from build123d import *

# Parameters (mm, degrees)
SKETCH_1_W          = 295
SKETCH_1_H          = 2005
EXTRUDE_1_DEPTH     = 30
SHELL_1_T           = -2
SKETCH_2_W          = 2
SKETCH_2_H          = 1467
EXTRUDE_2_DEPTH     = 220
SKETCH_3_R          = 4.5
CUT_EXTRUDE_1_DEPTH = 10
SKETCH_4_R          = 4.5
CUT_EXTRUDE_2_DEPTH = 116
SKETCH_5_R          = 4.5
CUT_EXTRUDE_3_DEPTH = 72
SKETCH_6_R          = 4.5
CUT_EXTRUDE_4_DEPTH = 10
CUT_EXTRUDE_START   = -10
SKETCH_7_R          = 4.5
CUT_EXTRUDE_5_DEPTH = 10
SKETCH_8_R          = 4.5
CUT_EXTRUDE_6_DEPTH = 16


with BuildPart() as part:
    # 草图1 → 凸台-拉伸1 (new body)
    with BuildSketch(Plane.XY):
        with Locations((147.5, 1002.5)):
            Rectangle(SKETCH_1_W, SKETCH_1_H)
    extrude(amount=EXTRUDE_1_DEPTH)

    # 抽壳1
    shell_1_openings = [part.faces().sort_by_distance(p)[0] for p in [
        (147.5, 1002.5, 30),
    ]]
    offset(amount=SHELL_1_T, openings=shell_1_openings, kind=Kind.INTERSECTION)

    # 草图2 → 凸台-拉伸2 (add)
    with BuildSketch(Plane.XY.offset(30)):
        with Locations((1, 773.5)):
            Rectangle(SKETCH_2_W, SKETCH_2_H)
    extrude(amount=EXTRUDE_2_DEPTH)

    # 草图3 → 切除-拉伸1 (cut)
    with BuildSketch(Plane(origin=(0, 2, 0), x_dir=(1, 0, 0), z_dir=(0, 1, 0))):
        with Locations(Location((30, -16, 0), (0, 0, 270))):
            Circle(SKETCH_3_R)
        with Locations(Location((200, -16, 0), (0, 0, 270))):
            Circle(SKETCH_3_R)
    extrude(amount=-CUT_EXTRUDE_1_DEPTH, mode=Mode.SUBTRACT)

    # 草图4 → 切除-拉伸2 (cut)
    with BuildSketch(Plane(origin=(2, 0, 0), x_dir=(0, 0, -1), z_dir=(1, 0, 0))):
        with Locations((-16, 30)):
            Circle(SKETCH_4_R)
        with Locations((-16, 180)):
            Circle(SKETCH_4_R)
    extrude(amount=-CUT_EXTRUDE_2_DEPTH, mode=Mode.SUBTRACT)

    # 草图5 → 切除-拉伸3 (cut)
    with BuildSketch(Plane(origin=(2, 0, 0), x_dir=(0, 0, -1), z_dir=(1, 0, 0))):
        with Locations((-16, 1975)):
            Circle(SKETCH_5_R)
        with Locations((-16, 1563)):
            Circle(SKETCH_5_R)
    extrude(amount=-CUT_EXTRUDE_3_DEPTH, mode=Mode.SUBTRACT)

    # 草图6 → 切除-拉伸4 (cut)
    with BuildSketch(Plane(origin=(0, 2005, 0), x_dir=(1, 0, 0), z_dir=(0, 1, 0))):
        with Locations(Location((30, -16, 0), (0, 0, 270))):
            Circle(SKETCH_6_R)
        with Locations(Location((265, -16, 0), (0, 0, 270))):
            Circle(SKETCH_6_R)
    extrude(amount=-CUT_EXTRUDE_4_DEPTH, mode=Mode.SUBTRACT)

    # 草图7 → 切除-拉伸5 (cut)
    with BuildSketch(Plane.ZY.offset(-293).offset(CUT_EXTRUDE_START)):
        with Locations(Location((16, 1975, 0), (0, 0, 180))):
            Circle(SKETCH_7_R)
        with Locations((16, 1676)):
            Circle(SKETCH_7_R)
        with Locations((16, 1377)):
            Circle(SKETCH_7_R)
        with Locations((16, 1317)):
            Circle(SKETCH_7_R)
        with Locations((16, 776)):
            Circle(SKETCH_7_R)
        with Locations((16, 235)):
            Circle(SKETCH_7_R)
    extrude(amount=CUT_EXTRUDE_5_DEPTH, mode=Mode.SUBTRACT)

    # 草图8 → 切除-拉伸6 (cut)
    with BuildSketch(Plane(origin=(295, 0, 0), x_dir=(0, 0, -1), z_dir=(1, 0, 0))):
        with Locations((-16, 30)):
            Circle(SKETCH_8_R)
        with Locations((-16, 175)):
            Circle(SKETCH_8_R)
    extrude(amount=-CUT_EXTRUDE_6_DEPTH, mode=Mode.SUBTRACT)


solid = part.part
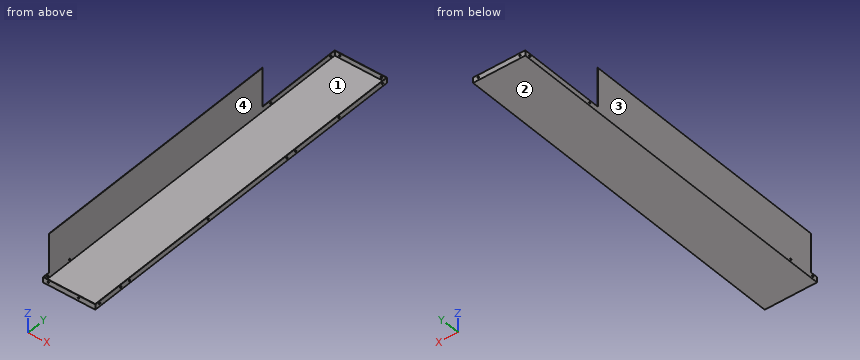
Build history of the part. All positions in model axes, mm. Face numbers are marked on the shaded views. A direction names the side the tool comes from. Round coordinates to 2 decimals unless told otherwise and drop trailing zeros. Write each loop counter-clockwise with the first axis right and the second up, starting at its lowest first coordinate (ties: lowest second). Pieces come first, ordered by that corner, then holes. Notation, with made-up numbers: M 78,-7.75 L 103,-7.75 A26 ccw 103,10.25 Z; hole C -10,9 d3. An arc over 180 degrees is marked long. Use CSV: the item, a comma, the result in double quotes.
1. Two-plate mould, pull along Y, no slides. Class the marked faces 1 and 2: +Y half, -Y half, draft (parallel to the pull), parting line (faces both ways), or undercut.
Reply:
face 1,"undercut"
face 2,"draft"
2. Wall check: probe 1 along Z at (x, y) = (293.9, 235); probe 2 along Z at (x, y) = (144.5, 956). Give the ranges that are in metal, low to high. Write a range as from..to.
Reply:
probe 1,"z = 0..11.5, 20.5..30"
probe 2,"z = 0..2"
3. Flat gauge pins, fed straight in: pin 1 (12 mm diameter, centred on x = 122.5, y = 657.5, fed in from +Z); pin 2 (0.6 mm diameter, centred on x = 1, z = 187, fed in from -Y); pin 3 (5.5 mm diameter, centred on x = 200, z = 16, fed in from -Y). Where does each tip first touch, or does it go through?
Reply:
pin 1,"stops at z = 2"
pin 2,"stops at y = 40"
pin 3,"stops at y = 2003"
4. Saw through at B-B (z = 156). Give the cut face in (x, y).
Reply:
outline,"M 0,40 L 2,40 L 2,1507 L 0,1507 Z"
5. Saw through at A-A (y = 942). Give the cut face in (x, z), plus the area to 3 significant figures.
Reply:
outline,"M 0,0 L 295,0 L 295,30 L 293,30 L 293,2 L 2,2 L 2,250 L 0,250 Z"
area,"1,140 mm²"
6. Tool access for the marked faces 3 and 4: list every direction of +Z, -Z, +X, -X, +Y, -Y with a clear straight run to the whole face (end or side of a thin tool).
Reply:
face 3,"+Z, -Z, -X, +Y, -Y"
face 4,"+Z"
